```python
from build123d import *

# Parameters (mm, degrees)
SKETCH_1_W          = 30
SKETCH_1_H          = 280
EXTRUDE_1_DEPTH     = 5
SKETCH_2_W          = 15
SKETCH_2_H          = 270
CUT_EXTRUDE_1_DEPTH = 142.155942135
FILLET_1_R          = 3
HOLE_WIZARD_M6_1_D  = 6.6
CHAMFER_1_SIZE      = 5
HOLE_WIZARD_M6_2_D  = 6.6
CHAMFER_2_SIZE      = 0.5
F_5_0MM_1_D         = 5
F_5_0MM_1_DEPTH     = 6
F_5_0MM_1_TIP       = 1.502151548


with BuildPart() as part:
    # 草图1 → 凸台-拉伸1 (new, symmetric)
    with BuildSketch(Plane.XY):
        Rectangle(SKETCH_1_W, SKETCH_1_H)
    extrude(amount=EXTRUDE_1_DEPTH, both=True)

    # 草图2 → 切除-拉伸1 (cut, through all)
    with BuildSketch(Plane(origin=(0, 0, -5), x_dir=(-1, 0, 0), z_dir=(0, 0, -1))):
        with Locations((-7.5, -5)):
            Rectangle(SKETCH_2_W, SKETCH_2_H)
    extrude(amount=-CUT_EXTRUDE_1_DEPTH, mode=Mode.SUBTRACT)

    # 圆角1
    fillet_1_edges = [part.edges().sort_by_distance(p)[0] for p in [
        (0, 130, 0),
    ]]
    fillet(fillet_1_edges, radius=FILLET_1_R)

    # M6 间隙孔1 (through all)
    with Locations(Plane(origin=(0, 130, 0), x_dir=(-1, 0, 0), z_dir=(0, -1, 0))):
        with Locations((-9, 0)):
            Hole(HOLE_WIZARD_M6_1_D / 2)

    # 倒角1
    chamfer_1_edges = [part.edges().sort_by_distance(p)[0] for p in [
        (0, -140, 0),
    ]]
    chamfer(chamfer_1_edges, length=CHAMFER_1_SIZE)

    # M6 间隙孔2 (through all)
    with Locations(Plane(origin=(0, 0, 0), x_dir=(0, 0, -1), z_dir=(1, 0, 0))):
        with Locations((0, 85), (0, 15), (0, -55), (0, -125)):
            Hole(HOLE_WIZARD_M6_2_D / 2)

    # 倒角2
    chamfer_2_edges = [part.edges().sort_by_distance(p)[0] for p in [
        (-15, 0, 5),
        (-10, -140, 5),
        (15, 135, -5),
        (15, 135, 5),
        (15, 130, 0),
        (9, 130, -5),
        (9, 130, 5),
        (0.878679656, 129.121320344, -5),
        (0.878679656, 129.121320344, 5),
        (0, -4, -5),
        (0, -4, 5),
        (-2.5, -137.5, -5),
        (-10, -140, -5),
        (-2.5, -137.5, 5),
        (-15, 0, -5),
        (0, 140, -5),
        (0, 140, 5),
        (-15, -140, 0),
        (-15, 140, 0),
        (15, 140, 0),
    ]]
    chamfer(chamfer_2_edges, length=CHAMFER_2_SIZE)

    # Ø5.0mm 暗销孔1
    with Locations(Plane(origin=(0, 140, 0), x_dir=(1, 0, 0), z_dir=(0, 1, 0))):
        with Locations((-9, 0)):
            Hole(F_5_0MM_1_D / 2, depth=F_5_0MM_1_DEPTH)
            with Locations((0, 0, -(F_5_0MM_1_DEPTH + F_5_0MM_1_TIP / 2))):  # 118° drill point
                Cone(0, F_5_0MM_1_D / 2, F_5_0MM_1_TIP, mode=Mode.SUBTRACT)


solid = part.part
```
Source: CAD feature listing. Evaluate the final solid. Frame: model axes, mm. A direction names the side the tool comes from. Coordinates: 2 decimals unless noted, no trailing zeros. Loops run counter-clockwise (first coordinate to the right, second up) from the corner with the lowest first, then second, coordinate; pieces in that order, holes last. Notation, with made-up numbers: M 73.25,-32 L 84.25,-32 A29 ccw 84.25,4 Z; hole C 18,61.25 d3. An arc over 180 degrees is marked long. Use a Markdown table: item, result. Add a question column.
Q1. Section query B-B, the plane y = -55. Return loops of the section in (x, z), and give its area (3 significant figures).
Q2. Material intervals for L1, parallel to Y at x = -6, z = 0; L2, parallel to Y at x = -7, z = -2.25; L3, parallel to Y at x = 7, z = 4, sorted ascending.
Q3. Section query C-C, the plane y = 70.5. Return loops of the section in (x, z).
Q4. Access query for faces 1 (the flat face through (0, -6, 0)), 2 (the cylindrical face through (-7.61, 17.23, -2.43)). Directions: +Z, -Z, +X, -X, +Y, -Y. A direction counts if a zero-diameter tool reaches every point of the face in a straight line with its end or side. Return the directions, or none.
Q5. Draft query along Z for faces 3 (the flat face through (-7, 2, 5)), 4 (the cylindrical face through (-6.5, 137, -0.1)), 5 (the flat face through (6, 130, -2)). Return one class per face: pulls with the +Z half, pulls with the -Z half, needs draft (parallel to the pull), parting line crosses it, or undercut.
Q6. Section query A-A, the plane x = 9. Return loops of the section in (y, z).
Q7. First-contact query: pin 1 (4.5 mm diameter, centred on x = 8, z = 1.5, fed in from -Y); pin 2 (5 mm diameter, centred on y = -77, z = 1.5, fed in from +X); pin 3 (5.5 mm diameter, centred on y = -125, z = 0, fed in from -X). Flat tips, straight axial feed; report the tip coordinate or a pass-through.
Result:
| question | item | result |
|---|---|---|
| 1 | outline | M -15,-4.5 L -14.5,-5 L -0.5,-5 L 0,-4.5 L 0,-3.3 L -15,-3.3 Z; M -15,3.3 L 0,3.3 L 0,4.5 L -0.5,5 L -14.5,5 L -15,4.5 Z |
| 1 | area | 50.5 mm2 |
| 2 | L1 | y = -140 to -128.3, -121.7 to -58.3, -51.7 to 11.7, 18.3 to 81.7, 88.3 to 140 |
| 2 | L2 | y = -140 to -127.41, -122.59 to -57.41, -52.59 to 12.59, 17.41 to 82.59, 87.41 to 140 |
| 2 | L3 | y = 130 to 140 |
| 3 | outline | M -15,-4.5 L -14.5,-5 L -0.5,-5 L 0,-4.5 L 0,4.5 L -0.5,5 L -14.5,5 L -15,4.5 Z |
| 4 | face 1 | +Z, -Z, +X, -Y |
| 4 | face 2 | +X, -X |
| 5 | face 3 | pulls with the +Z half |
| 5 | face 4 | undercut |
| 5 | face 5 | needs draft |
| 6 | outline | M 130,-4.5 L 130.5,-5 L 139.5,-5 L 140,-4.5 L 140,-3.3 L 130,-3.3 Z; M 130,3.3 L 140,3.3 L 140,4.5 L 139.5,5 L 130.5,5 L 130,4.5 Z |
| 7 | pin 1 | stops at y = 130 |
| 7 | pin 2 | stops at x = 0 |
| 7 | pin 3 | passes through |
